from build123d import *

# Parameters (mm, degrees)
SKETCH1_W           = 36
SKETCH1_H           = 8
BOSS_EXTRUDE1_DEPTH = 2
SKETCH2_R           = 1.75
CUT_EXTRUDE1_DEPTH  = 37.932370625
SKETCH3_R           = 4
BOSS_EXTRUDE2_DEPTH = 3
CHAMFER1_SIZE       = 0.5
CHAMFER2_SIZE       = 2


with BuildPart() as part:
    # Sketch1 → Boss-Extrude1 (new body)
    with BuildSketch(Plane(origin=(0, 0, 0), x_dir=(1, 0, 0), z_dir=(0, 1, 0))):
        with Locations((18, 4)):
            Rectangle(SKETCH1_W, SKETCH1_H)
    extrude(amount=BOSS_EXTRUDE1_DEPTH)

    # Sketch2 → Cut-Extrude1 (cut, through all)
    with BuildSketch(Plane(origin=(0, 2, 0), x_dir=(1, 0, 0), z_dir=(0, 1, 0))):
        with Locations(Location((5, 4, 0), (0, 0, 270))):
            Circle(SKETCH2_R)
    extrude(amount=-CUT_EXTRUDE1_DEPTH, mode=Mode.SUBTRACT)

    # Sketch3 → Boss-Extrude2 (add)
    with BuildSketch(Plane(origin=(0, 2, 0), x_dir=(1, 0, 0), z_dir=(0, 1, 0))):
        with Locations(Location((32, 4, 0), (0, 0, 270))):
            Circle(SKETCH3_R)
    extrude(amount=BOSS_EXTRUDE2_DEPTH)

    # Chamfer1
    chamfer1_edges = [part.edges().sort_by_distance(p)[0] for p in [
        (32, 5, -8),
    ]]
    chamfer(chamfer1_edges, length=CHAMFER1_SIZE)

    # Chamfer2
    chamfer2_edges = [part.edges().sort_by_distance(p)[0] for p in [
        (0, 1, -8),
        (36, 1, -8),
        (36, 1, 0),
        (0, 1, 0),
    ]]
    chamfer(chamfer2_edges, length=CHAMFER2_SIZE)


solid = part.part
Read the model definition and answer for the solid it produces. Units are mm, in the model's axes. A direction names the side the tool comes from. Round coordinates to 2 decimals unless told otherwise and drop trailing zeros. Loops run counter-clockwise (first coordinate to the right, second up) from the corner with the lowest first, then second, coordinate; pieces in that order, holes last.
Q1. Section C-C on x = 15.5 is taken. Write down the section's boundary in (y, z).
Q2. Section B-B on y = 0.4 is taken. Write down the section's boundary in (x, z), and give its area (3 significant figures).
Q3. Which of the six approach directions +Z, -Z, +X, -X, +Y, -Y give full straight-line access (tool end or side, diameter ignored) to faces 1 (the face through (18, 1, 0)), 2 (the face through (35.966, 3.232, -4.521))?
Q4. Consider probe 1 along X at (y, z) = (0.45, -4); probe 2 along Y at (x, z) = (7.5, -1); probe 3 along X at (y, z) = (4.3, -4). Determine where each line is inside the solid, lowest interval first.
Q5. Section A-A on x = 5 is taken. Write down the section's boundary in (y, z).
Q6. Each of these flat-tipped pins is pushed along its axis until it touches: pin 1 (1 mm diameter, centred on x = 18, z = -1, fed in from -Y); pin 2 (1.5 mm diameter, centred on y = 0.5, z = -7, fed in from -X). Where does it stop, or does it pass through?
Q7. Determine the mould class of faces 3 (the face through (36, 1, -4)), 4 (the face through (35, 1, -1)), 5 (the face through (3.94, 1.01, -5.39)), 6 (the face through (35, 1, -7)) for opening direction Z: released by +Z, released by -Z, zero draft, split by the parting line, or undercut.
Output:
1. outline: (0, -8) - (2, -8) - (2, 0) - (0, 0) - close
2. outline: (0, -6) - (2, -8) - (34, -8) - (36, -6) - (36, -2) - (34, 0) - (2, 0) - (0, -2) - close; hole circle Ø3.5 at (5, -4)
2. area: 270 mm2
3. face 1: +Z, +X, -X, +Y, -Y
3. face 2: +Y
4. probe 1: x = 0 to 3.25, 6.75 to 36
4. probe 2: y = 0 to 2
4. probe 3: x = 28 to 36
5. outline: (0, -8) - (2, -8) - (2, -5.75) - (0, -5.75) - close; (0, -2.25) - (2, -2.25) - (2, 0) - (0, 0) - close
6. pin 1: stops at y = 0
6. pin 2: stops at x = 0.25
7. face 3: zero draft
7. face 4: released by +Z
7. face 5: undercut
7. face 6: released by -Z
